Verification items for the finished model (mm, model axes). Give positions to 0.01 mm unless a question says otherwise; leave off trailing zeros. Write each loop counter-clockwise with the first axis right and the second up, starting at its lowest first coordinate (ties: lowest second). Pieces come first, ordered by that corner, then holes. Notation, with made-up numbers: (61.25, 29.5) - (116.25, 29.5) arc R29 ccw to (116.25, 68.5) - close; hole circle Ø10 at (-1.75, -8.75). An arc over 180 degrees is marked (long way). Answer as a JSON object with one key per item and string values. Group by question number.
Item 1: Sectioned sample at C-C, the plane y = -36.5. Record the boundary of the cut face in (x, z).
Item 2: Sectioned sample at D-D, the plane y = -22.5. Record the boundary of the cut face in (x, z), and give its area (3 significant figures).
Item 3: Scan lines: line 1 along X through (y, z) = (-5.5, 2.3); line 2 along X through (y, z) = (-27.5, 2.4); line 3 along X through (y, z) = (-32, 1). Record each from-to range of solid material in increasing order. Write a range as [from, to].
Item 4: Sectioned sample at B-B, the plane y = -11. Record the boundary of the cut face in (x, z), and give its area (3 significant figures).
Item 5: Sectioned sample at A-A, the plane z = 1.8. Record the boundary of the cut face in (x, y).
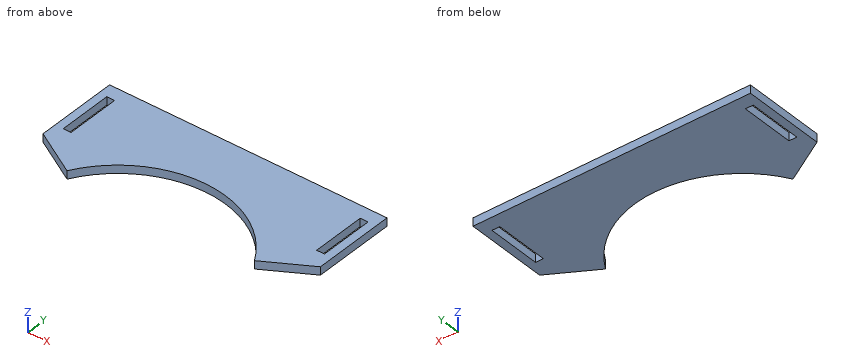
```python
from build123d import *

# Parameters (mm, degrees)
SKETCH1_W           = 2.9
SKETCH1_H           = 20
BOSS_EXTRUDE1_DEPTH = 3
CUT_EXTRUDE1_DEPTH  = 113.383299562


with BuildPart() as part:
    # Sketch1 → Boss-Extrude1 (new body)
    with BuildSketch(Plane.XY):
        with BuildLine():
            Line((0, 0), (104.9, 0))
            Line((104.9, 0), (104.9, -30))
            Line((104.9, -30), (87.212489335, -40.211889044))
            ThreePointArc((87.212489335, -40.211889044), (52.45, -20), (17.687510665, -40.211889044))
            Line((17.687510665, -40.211889044), (0, -30))
            Line((0, -30), (0, 0))
        make_face()
        with Locations((99.45, -15)):
            Rectangle(SKETCH1_W, SKETCH1_H, mode=Mode.SUBTRACT)
        with Locations((5.45, -15)):
            Rectangle(SKETCH1_W, SKETCH1_H, mode=Mode.SUBTRACT)
    extrude(amount=BOSS_EXTRUDE1_DEPTH)

    # Sketch2 → Cut-Extrude1 (cut, through all)
    with BuildSketch(Plane.XY.offset(3)):
        Polygon((1, 0), (1, -30.577350269), (0, -30), (0, 0), align=None)
        Polygon((103.9, 0), (103.9, -30.577350269), (104.9, -30), (104.9, 0), align=None)
    extrude(amount=-CUT_EXTRUDE1_DEPTH, mode=Mode.SUBTRACT)


solid = part.part
```
Geometry check:
{
 "1": {"outline": "(11.26, 0) - (20.08, 0) - (20.08, 3) - (11.26, 3) - close; (84.82, 0) - (93.64, 0) - (93.64, 3) - (84.82, 3) - close"},
 "2": {"outline": "(1, 0) - (4, 0) - (4, 3) - (1, 3) - close; (6.9, 0) - (38.53, 0) - (38.53, 3) - (6.9, 3) - close; (66.37, 0) - (98, 0) - (98, 3) - (66.37, 3) - close; (100.9, 0) - (103.9, 0) - (103.9, 3) - (100.9, 3) - close", "area": "208 mm^2"},
 "3": {"line 1": "[1, 4], [6.9, 98], [100.9, 103.9]", "line 2": "[1, 29.13], [75.77, 103.9]", "line 3": "[3.46, 23.88], [81.02, 101.44]"},
 "4": {"outline": "(1, 0) - (4, 0) - (4, 3) - (1, 3) - close; (6.9, 0) - (98, 0) - (98, 3) - (6.9, 3) - close; (100.9, 0) - (103.9, 0) - (103.9, 3) - (100.9, 3) - close", "area": "291 mm^2"},
 "5": {"outline": "(1, -30.58) - (17.69, -40.21) arc R40 cw to (87.21, -40.21) - (103.9, -30.58) - (103.9, 0) - (1, 0) - close; hole (4, -25) - (6.9, -25) - (6.9, -5) - (4, -5) - close; hole (98, -25) - (100.9, -25) - (100.9, -5) - (98, -5) - close"}
}
